Geometry: see drawing. Coordinates: mm, zero at the bounding-box minimum. A direction names the side the tool comes from. Coordinates: 2 decimals unless noted, no trailing zeros. Loops run counter-clockwise (first coordinate to the right, second up) from the corner with the lowest first, then second, coordinate; pieces in that order, holes last. Notation, with made-up numbers: M 52.5,1.25 L 96.5,1.25 A26 ccw 96.5,15.25 Z; hole C 76,14.5 d2. An arc over 180 degrees is marked long. One line per question, with ' | ' between items. Start each with the question number.
1. Mould query, pull axis X, two halves, no side actions, for the marked faces 1, 2 and 3. Classes: pulls with the +X half, pulls with the -X half, needs draft (parallel to the pull), parting line crosses it, or undercut.
2. Section query C-C, the plane x = 2.35. Output: boundary loops of the cut face in (y, z).
3. Ray query, probe 1 along X at (y, z) = (11, 3); probe 2 along Y at (x, z) = (2.65, 5.1); probe 3 along Y at (x, z) = (4, 2.6). Return the intervals inside material, ascending.
4. Section query D-D, the plane y = 3.75. Output: boundary loops of the cut face in (x, z).
5. Section query B-B, the plane y = 2.25. Output: boundary loops of the cut face in (x, z), and give its area (3 significant figures).
6. Pin query (flat end, axial travel): P1, Ø3, axis at y = 5.5, z = 4, coming from the +X side. Return the tip coordinate at first contact, or that it passes through.
7. Access query for the marked faces 4, 5 and 6. Directions: +Z, -Z, +X, -X, +Y, -Y. A direction counts if a zero-diameter tool reaches every point of the face in a straight line with its end or side. Return the directions, or none.
8. Section query A-A, the plane z = 3.55. Output: boundary loops of the cut face in (x, y) (1 decimal).
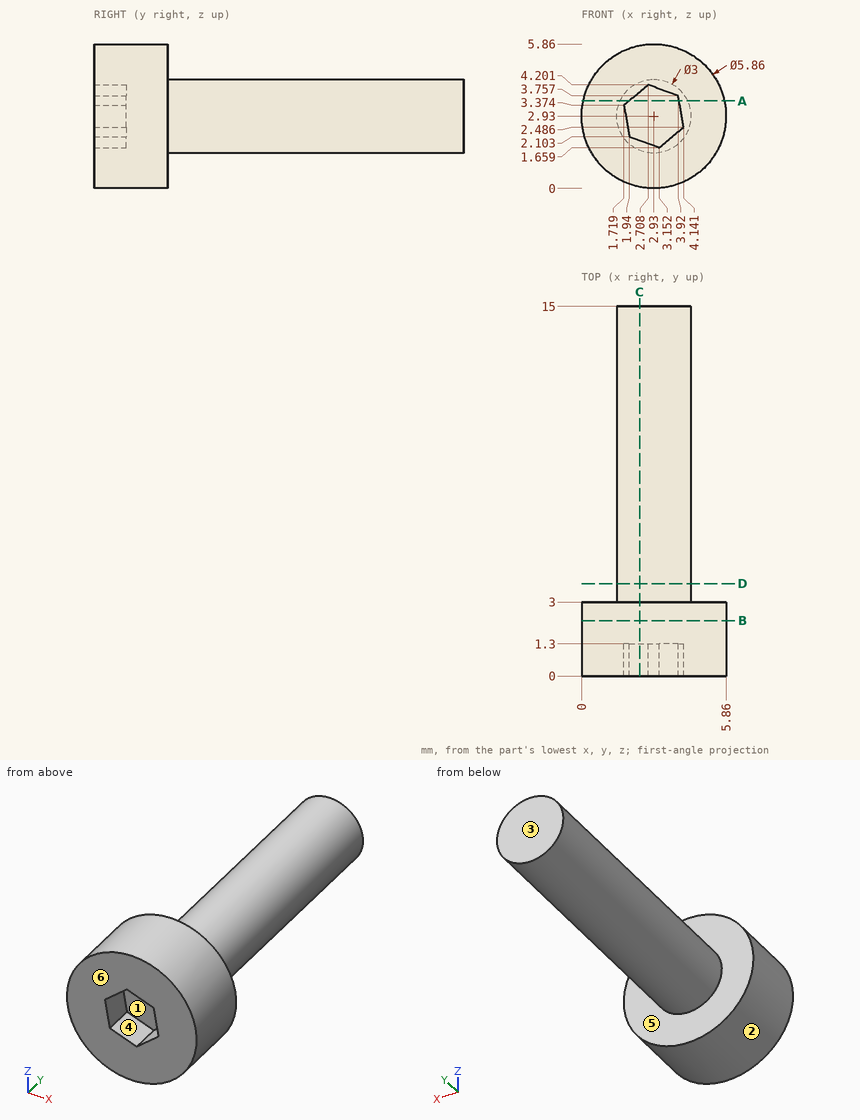
Taken from the geometry:
1) face 1: undercut | face 2: parting line crosses it | face 3: needs draft
2) outline: M 0,0.06 L 3,0.06 L 3,1.55 L 15,1.55 L 15,4.31 L 3,4.31 L 3,5.8 L 0,5.8 L 0,3.9 L 1.3,3.9 L 1.3,1.95 L 0,1.95 Z
3) probe 1: 1.43 to 4.43 | probe 2: 0 to 3 | probe 3: 1.3 to 15
4) outline: C 2.93,2.93 d3
5) outline: C 2.93,2.93 d5.86 | area: 27.0 mm^2
6) P1: x = 4.43
7) face 4: -Y | face 5: +Y | face 6: +Z, -Z, +X, -X, -Y
8) outline: M 0.1,0 L 1.9,0 L 1.9,1.3 L 4,1.3 L 4,0 L 5.8,0 L 5.8,3 L 4.3,3 L 4.3,15 L 1.6,15 L 1.6,3 L 0.1,3 Z
